The figure shows three views and two pictorial views of one solid part (mm, origin at its lowest corner). Answer the questions. Round coordinates to 2 decimals unless told otherwise and drop trailing zeros. Order: outer loops, then holes, each group sorted by start corner. A loop starts at its lowest first (then second) coordinate and runs counter-clockwise, first axis right, second up. Notation, with made-up numbers: (-33, 33) - (-14, 33) arc R21 ccw to (-14, 69) - close; hole circle Ø3 at (-2, 44). An arc over 180 degrees is marked (long way). Answer in a Markdown table with one row per item.
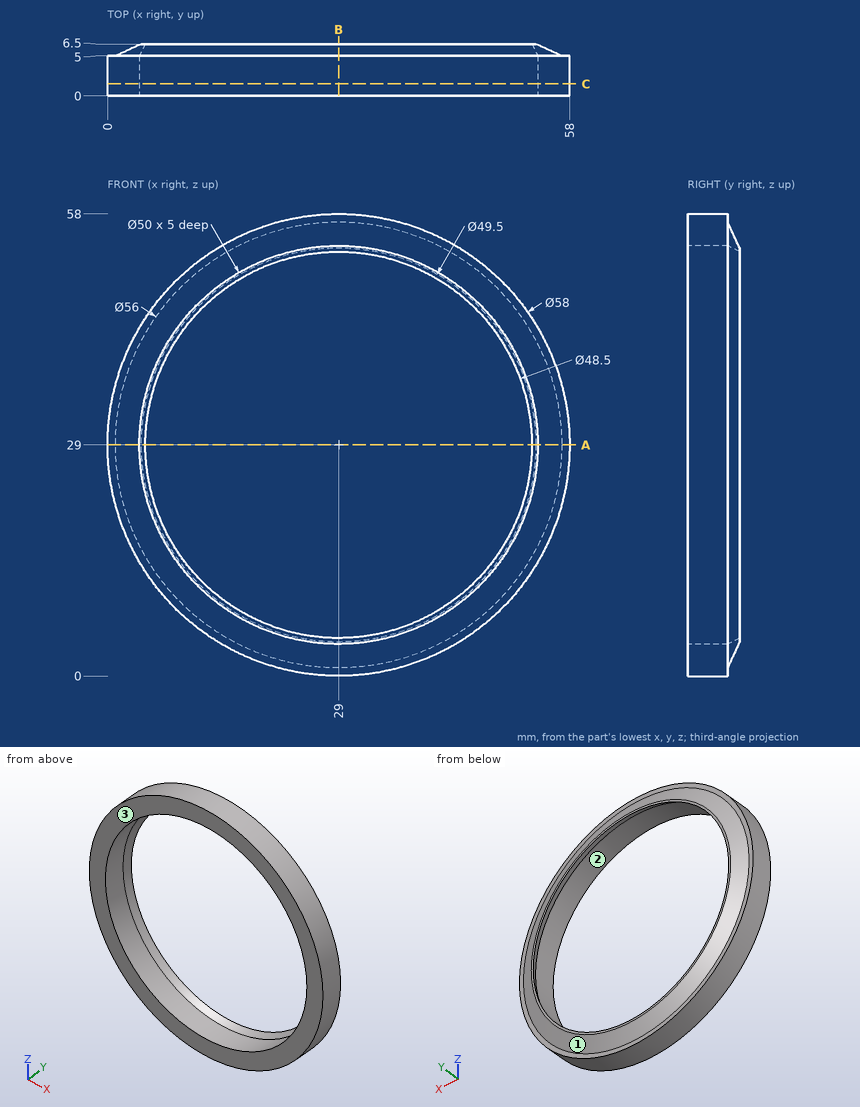
1) Find section C-C, the plane y = 1.5. Give the vertices of the cut face in (x, z).
Filled in:
| item | result |
|---|---|
| outline | circle Ø58 at (29, 29); hole circle Ø50 at (29, 29) |
2) Find the intervals of material crossed by probe 1 along X at (y, z) = (1.9, 29); probe 2 along Z at (x, y) = (44, 1.5), in increasing order. Write a range as from..to.
Filled in:
| item | result |
|---|---|
| probe 1 | x = 0..4, 54..58 |
| probe 2 | z = 4.18..9, 49..53.82 |
3) Find section A-A, the plane z = 29. Give the vertices of the cut face in (x, y), then the cut area to 4 significant figures.
Filled in:
| item | result |
|---|---|
| outline | (0, 0) - (4, 0) - (4, 5) - (4.75, 6.5) - (4.25, 6.5) - (1, 5) - (0, 5) - close; (53.25, 6.5) - (54, 5) - (54, 0) - (58, 0) - (58, 5) - (57, 5) - (53.75, 6.5) - close |
| area | 45.25 mm^2 |
4) Each of these flat-tipped pins is pushed along its axis until it touches: pin 1 (3 mm diameter, centred on y = 4, z = 10.5, fed in from -X); pin 2 (3 mm diameter, centred on x = 23, y = 1, fed in from +Z); pin 3 (17.5 mm diameter, centred on x = 20, z = 25, fed in from +Y); pin 4 (3 mm diameter, centred on x = 52, y = 2, fed in from -Z). Where does it stop, or does it pass through?
Filled in:
| item | result |
|---|---|
| pin 1 | stops at x = 5.51 |
| pin 2 | stops at z = 57.65 |
| pin 3 | passes through |
| pin 4 | stops at z = 9.54 |
5) The mould has two halves that part along Z. Classify the marked faces 1, 2 and 3: released by +Z, released by -Z, zero draft, split by the parting line, or undercut.
Filled in:
| item | result |
|---|---|
| face 1 | split by the parting line |
| face 2 | undercut |
| face 3 | zero draft |
6) Find section B-B, the plane x = 29. Give the vertices of the cut face in (y, z), then the cut area to 4 significant figures.
Filled in:
| item | result |
|---|---|
| outline | (0, 0) - (5, 0) - (5, 1) - (6.5, 4.25) - (6.5, 4.75) - (5, 4) - (0, 4) - close; (0, 54) - (5, 54) - (6.5, 53.25) - (6.5, 53.75) - (5, 57) - (5, 58) - (0, 58) - close |
| area | 45.25 mm^2 |
